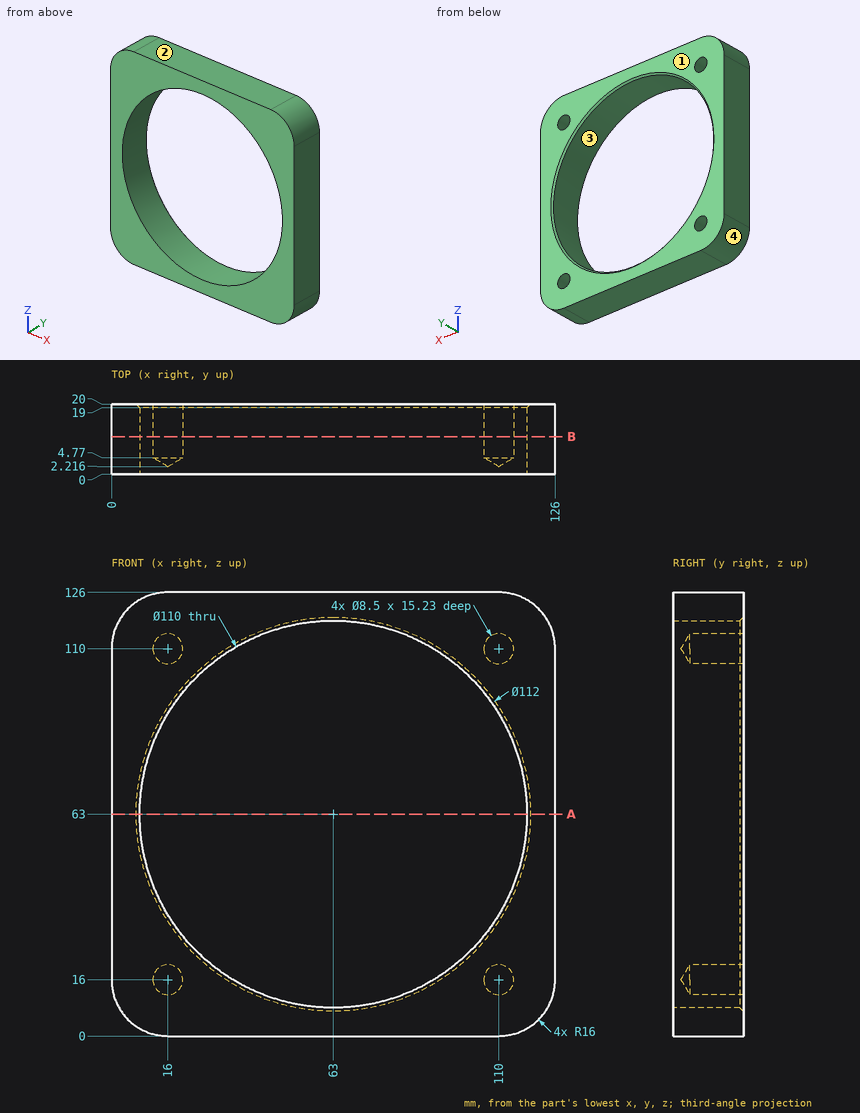
Job drawing, mm, ordinate dimensions from the low corner. One solid piece. Give positions to 0.01 mm unless a question says otherwise; leave off trailing zeros. Write each loop counter-clockwise with the first axis right and the second up, starting at its lowest first coordinate (ties: lowest second). Pieces come first, ordered by that corner, then holes. Notation, with made-up numbers: M -30.75,13 L -23.75,13 A24 cw -23.75,48 Z; hole C -21.75,82 d9. An arc over 180 degrees is marked long. One line per item, written item: value. Start each with the question number.
Q1. Drop a flat-ended pin along its axis: pin 1 Ø5 at (x, z) = (16, 16) entering from +Y. Give the stop position or say it passes through.
Q2. Two-plate mould, pull along Z, no slides. Class the marked faces 1, 2, 3 and 4: +Z half, -Z half, draft (parallel to the pull), parting line (faces both ways), or undercut.
Q3. Saw through at A-A, the plane z = 63. Write the cut outline in (x, y).
Q4. Saw through at B-B, the plane y = 10.75. Write the cut outline in (x, z).
Q5. Probe probe 1 along X at (y, z) = (15.25, 63.5); probe 2 along X at (y, z) = (15.25, 101); probe 3 along Z at (x, y) = (113, 14) (1 decimal). List the from-to ranges inside material, lowest first. Write a range as [from, to].
Output values:
1. pin 1: stops at y = 3.72
2. face 1: draft
2. face 2: +Z half
2. face 3: undercut
2. face 4: -Z half
3. outline: M 0,0 L 8,0 L 8,19 L 7,20 L 0,20 Z; M 118,0 L 126,0 L 126,20 L 119,20 L 118,19 Z
4. outline: M 0,16 A16 ccw 16,0 L 110,0 A16 ccw 126,16 L 126,110 A16 ccw 110,126 L 16,126 A16 ccw 0,110 Z; hole C 63,63 d110; hole C 16,16 d8.5; hole C 16,110 d8.5; hole C 110,16 d8.5; hole C 110,110 d8.5
5. probe 1: x = [0, 8], [118, 126]
5. probe 2: x = [0, 23.24], [102.76, 126]
5. probe 3: z = [0.3, 13], [19, 40.1], [85.9, 107], [113, 125.7]
